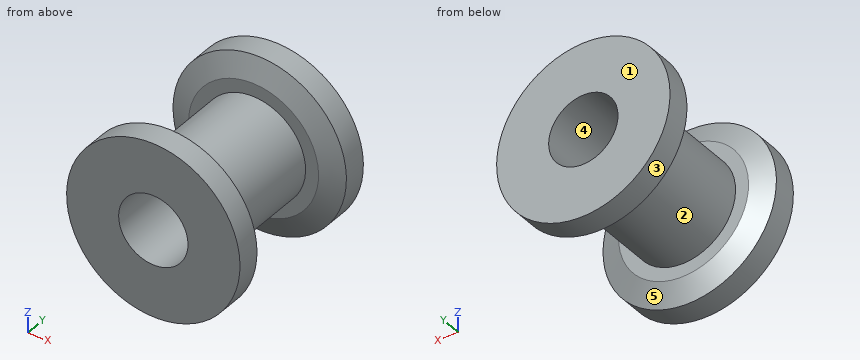
from build123d import *
from OCP.BRepFilletAPI import BRepFilletAPI_MakeChamfer

# Parameters (mm, degrees)
SKETCH1_R           = 20
SKETCH1_R_2         = 8
BOSS_EXTRUDE1_DEPTH = 40
SKETCH2_W           = 16
SKETCH2_H           = 25
CHAMFER1_SIZE       = 5
CHAMFER1_SIZE2      = 2


with BuildPart() as part:
    # Sketch1 → Boss-Extrude1 (new body)
    with BuildSketch(Plane(origin=(0, 0, 0), x_dir=(1, 0, 0), z_dir=(0, 1, 0))):
        with Locations(Location((0, 0, 0), (0, 0, 270))):
            Circle(SKETCH1_R)
        with Locations(Location((0, 0, 0), (0, 0, 270))):
            Circle(SKETCH1_R_2, mode=Mode.SUBTRACT)
    extrude(amount=BOSS_EXTRUDE1_DEPTH)

    # Sketch2 → Cut-Revolve1 (revolve, cut)
    with BuildSketch(Plane.XY, mode=Mode.PRIVATE) as cut_revolve1_sk:
        with Locations((20, 20)):
            Rectangle(SKETCH2_W, SKETCH2_H)
    revolve(cut_revolve1_sk.sketch.rotate(Axis((0, 0, 0), (0, 1, 0)), 90), axis=Axis((0, 0, 0), (0, 1, 0)), mode=Mode.SUBTRACT)

    # Chamfer1: one chamfer whose edges measure the first distance from different faces: ONE call of the kernel's chamfer builder (chamfer() names one face for all edges)
    chamfer1_edges_1 = [part.edges().sort_by_distance(p)[0] for p in [
        (0, 7.5, -20),
    ]]
    chamfer1_side_1 = [part.faces().sort_by_distance(p)[0] for p in [
        (0, 7.5, -19.434314575),
    ]]
    chamfer1_edges_2 = [part.edges().sort_by_distance(p)[0] for p in [
        (0, 32.5, -20),
    ]]
    chamfer1_side_2 = [part.faces().sort_by_distance(p)[0] for p in [
        (0, 32.5, -19.434314575),
    ]]
    chamfer1 = BRepFilletAPI_MakeChamfer(part.part.solid().wrapped)
    for e in chamfer1_edges_1:
        chamfer1.Add(CHAMFER1_SIZE, CHAMFER1_SIZE2, e.wrapped, chamfer1_side_1[0].wrapped)  # the first distance lies on this face
    for e in chamfer1_edges_2:
        chamfer1.Add(CHAMFER1_SIZE, CHAMFER1_SIZE2, e.wrapped, chamfer1_side_2[0].wrapped)  # the first distance lies on this face
    add(Compound.cast(chamfer1.Shape()), mode=Mode.REPLACE)


solid = part.part
Part model, mm, in its own coordinate system. Face numbers are marked on the shaded views. A direction names the side the tool comes from. Coordinates: 2 decimals unless noted, no trailing zeros. Loops run counter-clockwise (first coordinate to the right, second up) from the corner with the lowest first, then second, coordinate; pieces in that order, holes last. Notation, with made-up numbers: M -10.75,20.5 L 11.25,20.5 A20 cw 11.25,51.5 Z; hole C 73,-26 d4. An arc over 180 degrees is marked long. Use a Markdown table: item, result. Add a question column.
Q1. Cut at A-A (x = 0). Write the cut outline in (y, z), and give its area (3 significant figures).
Q2. Probe L1, parallel to X at y = 22.5, z = 0; L2, parallel to Y at x = 12, z = 1.5; L3, parallel to Z at x = -4, y = 18.5. List the from-to ranges inside material, lowest first.
Q3. Which spindle directions (+Z, -Z, +X, -X, +Y, -Y) get a long thin tool onto all of the face, cutting with end or side? Do the marked faces 4 and 5. Say none if no direction does.
Q4. Pin check, flat tips, straight feed: P1, Ø1, axis at y = 5, z = 3.5, coming from the -X side; P2, Ø1, axis at y = 5.5, z = 15.5, coming from the +X side. Stop position of each tip, or through.
Q5. Cut at B-B (z = 0). Write the cut outline in (x, y).
Q6. Mould opens along Y. For the marked faces 1, 2 and 3 say: +Y half, -Y half, draft (parallel to the pull), parting line (faces both ways), or undercut.
Q7. Cut at C-C (y = 23). Write the cut outline in (x, z).
Worked out:
| question | item | result |
|---|---|---|
| 1 | outline | M 0,-20 L 5.5,-20 L 7.5,-15 L 7.5,-12 L 32.5,-12 L 32.5,-15 L 34.5,-20 L 40,-20 L 40,-8 L 0,-8 Z; M 0,8 L 40,8 L 40,20 L 34.5,20 L 32.5,15 L 32.5,12 L 7.5,12 L 7.5,15 L 5.5,20 L 0,20 Z |
| 1 | area | 540 mm2 |
| 2 | L1 | x = -12 to -8, 8 to 12 |
| 2 | L2 | y = 0 to 7.5, 32.5 to 40 |
| 2 | L3 | z = -11.31 to -6.93, 6.93 to 11.31 |
| 3 | face 4 | +Y, -Y |
| 3 | face 5 | none |
| 4 | P1 | stops at x = -19.77 |
| 4 | P2 | stops at x = 13.23 |
| 5 | outline | M -20,0 L -8,0 L -8,40 L -20,40 L -20,34.5 L -15,32.5 L -12,32.5 L -12,7.5 L -15,7.5 L -20,5.5 Z; M 8,0 L 20,0 L 20,5.5 L 15,7.5 L 12,7.5 L 12,32.5 L 15,32.5 L 20,34.5 L 20,40 L 8,40 Z |
| 6 | face 1 | +Y half |
| 6 | face 2 | undercut |
| 6 | face 3 | draft |
| 7 | outline | C 0,0 d24; hole C 0,0 d16 |
